Design review of the part built by this model. Coordinates are the model's own, in mm. Give positions to 0.01 mm unless a question says otherwise; leave off trailing zeros.
```python
from build123d import *

# Parameters (mm, degrees)
EXTRUDE1_DEPTH      = 1081
EXTRUDE4_DEPTH      = 1083.285410341
EXTRUDE4_DEPTH_BACK = 1083.285410341
EXTRUDE5_DEPTH      = 30


with BuildPart() as part:
    # Sketch2 → Extrude1 (new body)
    with BuildSketch(Plane.XY):
        with BuildLine():
            Line((27.429618111, 61.203514875), (27.429618111, 62.483514875))
            Line((27.429618111, 62.483514875), (27.063725093, 65.097036429))
            ThreePointArc((27.063725093, 65.097036429), (26.9381678, 66.899458408), (27.063725093, 68.701880387))
            Line((27.063725093, 68.701880387), (27.290970266, 70.325060195))
            ThreePointArc((27.290970266, 70.325060195), (27.40740123, 70.522960701), (27.629667144, 70.580568366))
            Line((27.629667144, 70.580568366), (28.223872192, 70.497379659))
            ThreePointArc((28.223872192, 70.497379659), (28.421772697, 70.380948695), (28.479380362, 70.158682782))
            Line((28.479380362, 70.158682782), (28.252135189, 68.535502974))
            ThreePointArc((28.252135189, 68.535502974), (28.1381678, 66.899458408), (28.252135189, 65.263413843))
            Line((28.252135189, 65.263413843), (28.629618111, 62.56710726))
            Line((28.629618111, 62.56710726), (34.119618111, 62.56710726))
            Line((34.119618111, 62.56710726), (34.119618111, 64.76710726))
            Line((34.119618111, 64.76710726), (35.119618111, 64.76710726))
            ThreePointArc((35.119618111, 64.76710726), (36.498022986, 64.671651671), (37.850112572, 64.38710726))
            ThreePointArc((37.850112572, 64.38710726), (40.451975855, 64.047973934), (43.040517634, 64.47710726))
            Line((43.040517634, 64.47710726), (46.429618111, 65.567355231))
            Line((46.429618111, 65.567355231), (46.429618111, 64.306791917))
            Line((46.429618111, 64.306791917), (43.408001834, 63.334760831))
            ThreePointArc((43.408001834, 63.334760831), (40.472780352, 62.848154292), (37.522453236, 63.23270726))
            ThreePointArc((37.522453236, 63.23270726), (36.431587911, 63.468758554), (35.319618111, 63.564834239))
            Line((35.319618111, 63.564834239), (35.319618111, 62.56710726))
            Line((35.319618111, 62.56710726), (41.399618111, 62.56710726))
            ThreePointArc((41.399618111, 62.56710726), (44.228045236, 61.395534384), (45.399618111, 58.56710726))
            Line((45.399618111, 58.56710726), (45.399618111, 53.252873744))
            ThreePointArc((45.399618111, 53.252873744), (45.127835843, 52.807995483), (44.607951444, 52.846757313))
            ThreePointArc((44.607951444, 52.846757313), (41.599927405, 51.269233396), (44.662909839, 49.801265776))
            ThreePointArc((44.662909839, 49.801265776), (45.204517239, 49.836690545), (45.440067721, 49.347702344))
            ThreePointArc((45.440067721, 49.347702344), (45.673249329, 48.549369428), (46.429618111, 48.203514875))
            Line((46.429618111, 48.203514875), (24.429618111, 48.203514875))
            Line((24.429618111, 48.203514875), (24.429618111, 73.203514875))
            Line((24.429618111, 73.203514875), (26.429618111, 73.203514875))
            Line((26.429618111, 73.203514875), (26.429618111, 61.203514875))
            Line((26.429618111, 61.203514875), (27.429618111, 61.203514875))
        make_face()
    extrude(amount=EXTRUDE1_DEPTH)

    # Sketch4 → Extrude4 (cut, two sides: drawn at the far end of the back side and taken through both)
    with BuildSketch(Plane.XZ.offset(-48.203514875).offset(-EXTRUDE4_DEPTH_BACK)):
        Polygon((24.429618111, 0), (46.429618111, 0), (24.429618111, 22), align=None)
    extrude(amount=EXTRUDE4_DEPTH + EXTRUDE4_DEPTH_BACK, mode=Mode.SUBTRACT)

    # Sketch5 → Extrude5 (cut)
    with BuildSketch(Plane.XZ.offset(-48.203514875)):
        Polygon((46.429618111, 1081), (24.429618111, 1059), (24.429618111, 1081), align=None)
    extrude(amount=-EXTRUDE5_DEPTH, mode=Mode.SUBTRACT)


solid = part.part
```
(1) To check wall thickness, follow L1, parallel to Y at x = 42.25, z = 849.5; L2, parallel to X at y = 62, z = 751.5; L3, parallel to Y at x = 38, z = 504. State the ranges of each line that lie inside material, in increasing order.
Resolved:
L1: y = 48.2 to 49.87, 52.73 to 62.48, 63.04 to 64.26
L2: x = 24.43 to 26.43, 27.43 to 43.45
L3: y = 48.2 to 62.57, 63.11 to 64.35
(2) Mouldability with a two-part tool opening along X and no side actions: class faces 1 (the face through (36, 48.204, 533)), 2 (the face through (33.14, 57.75, 1067.71)) as pulls with the +X half, pulls with the -X half, needs draft (parallel to the pull), parting line crosses it, or undercut.
Resolved:
face 1: needs draft
face 2: pulls with the -X half
(3) Clearance check with flat-ended pins moving along their axes: P1, Ø2.5, axis at y = 55.5, z = 628, coming from the +X side; P2, Ø2, axis at x = 34.5, y = 52, coming from the +Z side; P3, Ø6, axis at x = 30.5, z = 748.5, coming from the +Y side. State where each tip first meets the part, or that it passes through.
Resolved:
P1: stops at x = 45.4
P2: stops at z = 1070.07
P3: stops at y = 70.58
